Check sheet for the modelled part. Datum: model origin and axes. Units: mm. A direction names the side the tool comes from. Coordinates: 2 decimals unless noted, no trailing zeros. Write each loop counter-clockwise with the first axis right and the second up, starting at its lowest first coordinate (ties: lowest second). Pieces come first, ordered by that corner, then holes. Notation, with made-up numbers: (21, 78.5) -> (35, 78.5) arc R18 cw to (35, 100.5) -> close; hole circle Ø1 at (0, 85). An arc over 180 degrees is marked (long way). Put each result on its own line as item: value.
```python
from build123d import *

# Parameters (mm, degrees)
CHAMFER1_SIZE           = 1
SKETCH3_W               = 5.79915747
SKETCH3_H               = 1.2
CUT_EXTRUDE2_DEPTH      = 181.865972477
CUT_EXTRUDE2_DEPTH_BACK = 181.865972477
SKETCH7_W               = 12.649467172
SKETCH7_H               = 42.427609508
CUT_EXTRUDE3_DEPTH      = 181.865972477
CUT_EXTRUDE3_DEPTH_BACK = 181.865972477
SKETCH8_W               = 5.603563882
SKETCH8_H               = 43.977481417


with BuildPart() as part:
    # Sketch1 → Revolve1 (revolve)
    with BuildSketch(Plane.XY, mode=Mode.PRIVATE) as revolve1_sk:
        Polygon((0, 180), (10, 180), (10, 45), (12.5, 45), (12.5, 25), (8, 25), (8, 0), (0, 0), align=None)
    revolve(revolve1_sk.sketch.rotate(Axis((0, 0, 0), (0, 1, 0)), 90), axis=Axis((0, 0, 0), (0, 1, 0)))

    # Chamfer1
    chamfer1_edges = [part.edges().sort_by_distance(p)[0] for p in [
        (0, 0, 8),
        (0, 180, 10),
    ]]
    chamfer(chamfer1_edges, length=CHAMFER1_SIZE)

    # Sketch3 → Cut-Revolve1 (revolve, cut)
    with BuildSketch(Plane.XY, mode=Mode.PRIVATE) as cut_revolve1_sk:
        with Locations((-12.399578735, 159.6)):
            Rectangle(SKETCH3_W, SKETCH3_H)
    revolve(cut_revolve1_sk.sketch.rotate(Axis((0, 180, 0), (0, -1, 0)), 270), axis=Axis((0, 180, 0), (0, -1, 0)), mode=Mode.SUBTRACT)

    # Sketch7 → Cut-Extrude2 (cut, two sides: drawn at the far end of the back side and taken through both)
    with BuildSketch(Plane.XY.offset(-CUT_EXTRUDE2_DEPTH_BACK)):
        with Locations((-14.824733586, 186.213804754)):
            Rectangle(SKETCH7_W, SKETCH7_H)
        with Locations((14.824733586, 186.213804754)):
            Rectangle(SKETCH7_W, SKETCH7_H)
    extrude(amount=CUT_EXTRUDE2_DEPTH + CUT_EXTRUDE2_DEPTH_BACK, mode=Mode.SUBTRACT)

    # Sketch8 → Cut-Extrude3 (cut, two sides: drawn at the far end of the back side and taken through both)
    with BuildSketch(Plane(origin=(0, 0, 0), x_dir=(0, 0, -1), z_dir=(1, 0, 0)).offset(-CUT_EXTRUDE3_DEPTH_BACK)):
        with Locations((-11.301781941, 186.988740709)):
            Rectangle(SKETCH8_W, SKETCH8_H)
        with Locations((11.301781941, 186.988740709)):
            Rectangle(SKETCH8_W, SKETCH8_H)
    extrude(amount=CUT_EXTRUDE3_DEPTH + CUT_EXTRUDE3_DEPTH_BACK, mode=Mode.SUBTRACT)


solid = part.part
```
Q1. Material ranges on line 1 along X through (y, z) = (28, 7.5); line 2 along Y through (x, z) = (5.5, 6.5); line 3 along Y through (x, z) = (0.25, -9.25), recorded low to high.
Recorded:
line 1: x = -10 to 10
line 2: y = 25 to 180
line 3: y = 25 to 165
Q2. Cross-section at C-C (y = 49). Record the cut outline in (x, z).
Recorded:
outline: circle Ø20 at (0, 0)
Q3. Depth check by flat-ended pin: P1, Ø11.5, axis at x = -1.5, y = 170, coming from the -Z side; P2, Ø1, axis at x = -2, z = -7, coming from the -Y side; P3, Ø1.6, axis at x = 0, z = -9.5, coming from the +Y side; P4, Ø6, axis at x = -2.5, y = 49.5, coming from the +Z side. Enter the tip coordinate at first touch or a pass-through.
Recorded:
P1: stops at z = -10
P2: stops at y = 0
P3: stops at y = 165
P4: stops at z = 10
Q4. Tool access check on faces 1 (the cylindrical face through (0, 101, 10)), 2 (the flat face through (8.5, 172, 0)), 3 (the cylindrical face through (5.78, 159.61, -7.54)). Record the directions out of +Z, -Z, +X, -X, +Y, -Y that give a thin tool (end or side, any length) a straight path to the whole face; none if there is none.
Recorded:
face 1: +Y
face 2: +Z, -Z, +X, +Y
face 3: none
Q5. Mould release check, pull along Y, two halves, no side actions. Record for faces 4 (the flat face through (4, 160.2, 9)), 5 (the flat face through (0, 172, -8.5)), 6 (the conical face through (-6.6, 179.6, -6.69)): released by +Y, released by -Y, zero draft, split by the parting line, or undercut.
Recorded:
face 4: undercut
face 5: zero draft
face 6: released by +Y
Q6. Cross-section at B-B (x = 0). Record the cut outline in (y, z).
Recorded:
outline: (0, -7) -> (1, -8) -> (25, -8) -> (25, -12.5) -> (45, -12.5) -> (45, -10) -> (159, -10) -> (159, -9.5) -> (160.2, -9.5) -> (160.2, -10) -> (165, -10) -> (165, -8.5) -> (180, -8.5) -> (180, 8.5) -> (165, 8.5) -> (165, 10) -> (160.2, 10) -> (160.2, 9.5) -> (159, 9.5) -> (159, 10) -> (45, 10) -> (45, 12.5) -> (25, 12.5) -> (25, 8) -> (1, 8) -> (0, 7) -> close
Q7. Cross-section at A-A (z = 0). Record the cut outline in (x, y), plus the area to 3 significant figures.
Recorded:
outline: (-12.5, 25) -> (-8, 25) -> (-8, 1) -> (-7, 0) -> (7, 0) -> (8, 1) -> (8, 25) -> (12.5, 25) -> (12.5, 45) -> (10, 45) -> (10, 159) -> (9.5, 159) -> (9.5, 160.2) -> (10, 160.2) -> (10, 165) -> (8.5, 165) -> (8.5, 180) -> (-8.5, 180) -> (-8.5, 165) -> (-10, 165) -> (-10, 160.2) -> (-9.5, 160.2) -> (-9.5, 159) -> (-10, 159) -> (-10, 45) -> (-12.5, 45) -> close
area: 3,550 mm2
